```python
from build123d import *

# Parameters (mm, degrees)
BRACKET_BODY_DEPTH      = 56
SLOT_SKETCH_W           = 62
SLOT_SKETCH_H           = 20
SLOT_CUT_DEPTH          = 90.112288715
LUG_A_SKETCH_R          = 32
LUG_A_SKETCH_R_2        = 18
LUG_A_14MM_DEPTH        = 14
SPACER_START            = 2
SPACER_A_SKETCH_R       = 32
SPACER_A_SKETCH_R_2     = 18
SPACER_A_2MM_DEPTH      = 2
HOLE_A_SKETCH_R         = 18
HOLE_A_DEPTH            = 107.244999882
SPACER_B_SKETCH_R       = 32
SPACER_B_SKETCH_R_2     = 18
SPACER_B_2MM_DEPTH      = 2
LUG_B_SKETCH_R          = 32
LUG_B_SKETCH_R_2        = 18
LUG_B_14MM_DEPTH        = 14
PAD_SKETCH_R            = 25
PAD_SKETCH_R_2          = 12.5
PAD_2MM_DEPTH           = 2
HUB_START               = -44
HUB_SKETCH_R            = 25
HUB_SKETCH_R_2          = 12.5
HUB_44MM_DEPTH          = 44
HUB_BORE_SKETCH_R       = 12.5
HUB_BORE_DEPTH          = 44
ARM_35MM_DEPTH          = 35
ARM_SPACER_A_SKETCH_R   = 17.5
ARM_SPACER_A_SKETCH_R_2 = 10
ARM_SPACER_A_2MM_DEPTH  = 2
ARM_START               = -12
ARM_LUG_SKETCH_R        = 17.5
ARM_LUG_SKETCH_R_2      = 10
ARM_LUG_12MM_DEPTH      = 12
ARM_HOLE_SKETCH_R       = 10
ARM_HOLE_DEPTH          = 150.390672563
ARM_SPACER_B_SKETCH_R   = 17.5
ARM_SPACER_B_SKETCH_R_2 = 10
ARM_SPACER_B_2MM_DEPTH  = 2
ARM_START_2             = -14
ARM_EYE_SKETCH_R        = 17.5
ARM_EYE_SKETCH_R_2      = 10
ARM_EYE_14MM_DEPTH      = 14
ARM_SLOT_SKETCH_W       = 12.731987003
ARM_SLOT_SKETCH_H       = 35
ARM_SLOT_10MM_DEPTH     = 10
PIN_START               = -16
PIN_BOSS_SKETCH_R       = 25
PIN_BOSS_16MM_DEPTH     = 16
PIN_BOSS_HOLE_SKETCH_R  = 12.5
PIN_BOSS_HOLE_DEPTH     = 151.168319402


with BuildPart() as part:
    # Bracket Profile Sketch → Bracket Body (new body)
    with BuildSketch(Plane.XY):
        Polygon((0, 0), (17, 0), (17, -48), (31, -48), (31, 12), (9, 12), (9, 62), (-9, 62), (-9, 12), (-31, 12), (-31, -48), (-17, -48), (-17, 0), align=None)
    extrude(amount=-BRACKET_BODY_DEPTH)

    # Slot Sketch → Slot Cut (cut, through all)
    with BuildSketch(Plane.XY):
        with Locations((0, -38)):
            Rectangle(SLOT_SKETCH_W, SLOT_SKETCH_H)
    extrude(amount=-SLOT_CUT_DEPTH, mode=Mode.SUBTRACT)

    # Lug A Sketch → Lug A 14mm (add)
    with BuildSketch(Plane(origin=(31, 0, 0), x_dir=(0, 0, -1), z_dir=(1, 0, 0))):
        with Locations((28, -28)):
            Circle(LUG_A_SKETCH_R)
        with Locations((28, -28)):
            Circle(LUG_A_SKETCH_R_2, mode=Mode.SUBTRACT)
    extrude(amount=-LUG_A_14MM_DEPTH)

    # Spacer A Sketch → Spacer A 2mm (add)
    with BuildSketch(Plane(origin=(31, 0, 0), x_dir=(0, 0, -1), z_dir=(1, 0, 0)).offset(SPACER_START)):
        with Locations(Location((28, -28, 0), (0, 0, 90))):
            Circle(SPACER_A_SKETCH_R)
        with Locations(Location((28, -28, 0), (0, 0, 90))):
            Circle(SPACER_A_SKETCH_R_2, mode=Mode.SUBTRACT)
    extrude(amount=-SPACER_A_2MM_DEPTH)

    # Hole A Sketch → Hole A (cut, through all)
    with BuildSketch(Plane(origin=(31, 0, 0), x_dir=(0, 0, -1), z_dir=(1, 0, 0))):
        with Locations(Location((28, -28, 0), (0, 0, 90))):
            Circle(HOLE_A_SKETCH_R)
    extrude(amount=-HOLE_A_DEPTH, mode=Mode.SUBTRACT)

    # Spacer B Sketch → Spacer B 2mm (add)
    with BuildSketch(Plane.ZY.offset(31)):
        with Locations(Location((-28, -28, 0), (0, 0, 90))):
            Circle(SPACER_B_SKETCH_R)
        with Locations(Location((-28, -28, 0), (0, 0, 90))):
            Circle(SPACER_B_SKETCH_R_2, mode=Mode.SUBTRACT)
    extrude(amount=SPACER_B_2MM_DEPTH)

    # Lug B Sketch → Lug B 14mm (add)
    with BuildSketch(Plane(origin=(-17, 0, 0), x_dir=(0, 0, -1), z_dir=(1, 0, 0))):
        with Locations(Location((28, -28, 0), (0, 0, 90))):
            Circle(LUG_B_SKETCH_R)
        with Locations(Location((28, -28, 0), (0, 0, 90))):
            Circle(LUG_B_SKETCH_R_2, mode=Mode.SUBTRACT)
    extrude(amount=-LUG_B_14MM_DEPTH)

    # Pad Sketch → Pad 2mm (add)
    with BuildSketch(Plane.ZY.offset(9)):
        with Locations(Location((-28, 50, 0), (0, 0, 151.314597986))):
            Circle(PAD_SKETCH_R)
        with Locations(Location((-28, 50, 0), (0, 0, 73.739795292))):
            Circle(PAD_SKETCH_R_2, mode=Mode.SUBTRACT)
    extrude(amount=PAD_2MM_DEPTH)

    # Hub Sketch → Hub 44mm (add)
    with BuildSketch(Plane.ZY.offset(11).offset(HUB_START)):
        with Locations(Location((-28, 50, 0), (0, 0, 270))):
            Circle(HUB_SKETCH_R)
        with Locations(Location((-28, 50, 0), (0, 0, 270))):
            Circle(HUB_SKETCH_R_2, mode=Mode.SUBTRACT)
    extrude(amount=HUB_44MM_DEPTH)

    # Hub Bore Sketch → Hub Bore (cut)
    with BuildSketch(Plane.ZY.offset(9).offset(HUB_START)):
        with Locations(Location((-28, 50, 0), (0, 0, 270))):
            Circle(HUB_BORE_SKETCH_R)
    extrude(amount=HUB_BORE_DEPTH, mode=Mode.SUBTRACT)

    # Arm Profile Sketch → Arm 35mm (add)
    with BuildSketch(Plane(origin=(0, 62, 0), x_dir=(1, 0, 0), z_dir=(0, 1, 0))):
        Polygon((3.731987003, 49.931712199), (3.731987003, 79.931712199), (-8.268012997, 79.931712199), (-8.268012997, 104.931712199), (3.731987003, 104.931712199), (3.731987003, 92.431712199), (18.731987003, 92.431712199), (18.731987003, 104.931712199), (30.731987003, 104.931712199), (30.731987003, 79.931712199), (18.731987003, 79.931712199), (18.731987003, 49.931712199), align=None)
    extrude(amount=-ARM_35MM_DEPTH)

    # Arm Spacer A Sketch → Arm Spacer A 2mm (add)
    with BuildSketch(Plane.ZY.offset(8.268012997)):
        with Locations(Location((-104.931712199, 44.5, 0), (0, 0, 270))):
            Circle(ARM_SPACER_A_SKETCH_R)
        with Locations(Location((-104.931712199, 44.5, 0), (0, 0, 90))):
            Circle(ARM_SPACER_A_SKETCH_R_2, mode=Mode.SUBTRACT)
    extrude(amount=ARM_SPACER_A_2MM_DEPTH)

    # Arm Lug Sketch → Arm Lug 12mm (add)
    with BuildSketch(Plane.ZY.offset(8.268012997).offset(ARM_START)):
        with Locations(Location((-104.931712199, 44.5, 0), (0, 0, 90))):
            Circle(ARM_LUG_SKETCH_R)
        with Locations(Location((-104.931712199, 44.5, 0), (0, 0, 90))):
            Circle(ARM_LUG_SKETCH_R_2, mode=Mode.SUBTRACT)
    extrude(amount=ARM_LUG_12MM_DEPTH)

    # Arm Hole Sketch → Arm Hole (cut, through all)
    with BuildSketch(Plane.ZY.offset(8.268012997)):
        with Locations((-104.931712199, 44.5)):
            Circle(ARM_HOLE_SKETCH_R)
    extrude(amount=-ARM_HOLE_DEPTH, mode=Mode.SUBTRACT)

    # Arm Spacer B Sketch → Arm Spacer B 2mm (add)
    with BuildSketch(Plane(origin=(30.731987003, 0, 0), x_dir=(0, 0, -1), z_dir=(1, 0, 0))):
        with Locations(Location((104.931712199, 44.5, 0), (0, 0, 90))):
            Circle(ARM_SPACER_B_SKETCH_R)
        with Locations(Location((104.931712199, 44.5, 0), (0, 0, 180))):
            Circle(ARM_SPACER_B_SKETCH_R_2, mode=Mode.SUBTRACT)
    extrude(amount=ARM_SPACER_B_2MM_DEPTH)

    # Arm Eye Sketch → Arm Eye 14mm (add)
    with BuildSketch(Plane(origin=(32.731987003, 0, 0), x_dir=(0, 0, -1), z_dir=(1, 0, 0)).offset(ARM_START_2)):
        with Locations(Location((104.931712199, 44.5, 0), (0, 0, 90))):
            Circle(ARM_EYE_SKETCH_R)
        with Locations(Location((104.931712199, 44.5, 0), (0, 0, 180))):
            Circle(ARM_EYE_SKETCH_R_2, mode=Mode.SUBTRACT)
    extrude(amount=ARM_EYE_14MM_DEPTH)

    # Arm Slot Sketch → Arm Slot 10mm (cut)
    with BuildSketch(Plane(origin=(0, 0, -56), x_dir=(-1, 0, 0), z_dir=(0, 0, -1))):
        with Locations((2.634006498, 44.5)):
            Rectangle(ARM_SLOT_SKETCH_W, ARM_SLOT_SKETCH_H)
    extrude(amount=-ARM_SLOT_10MM_DEPTH, mode=Mode.SUBTRACT)

    # Pin Boss Sketch → Pin Boss 16mm (add)
    with BuildSketch(Plane.ZY.offset(11).offset(PIN_START)):
        with Locations(Location((-28, 50, 0), (0, 0, 270))):
            Circle(PIN_BOSS_SKETCH_R)
    extrude(amount=PIN_BOSS_16MM_DEPTH)

    # Pin Boss Hole Sketch → Pin Boss Hole (cut, through all)
    with BuildSketch(Plane.ZY.offset(11)):
        with Locations(Location((-28, 50, 0), (0, 0, 270))):
            Circle(PIN_BOSS_HOLE_SKETCH_R)
    extrude(amount=-PIN_BOSS_HOLE_DEPTH, mode=Mode.SUBTRACT)


solid = part.part
```
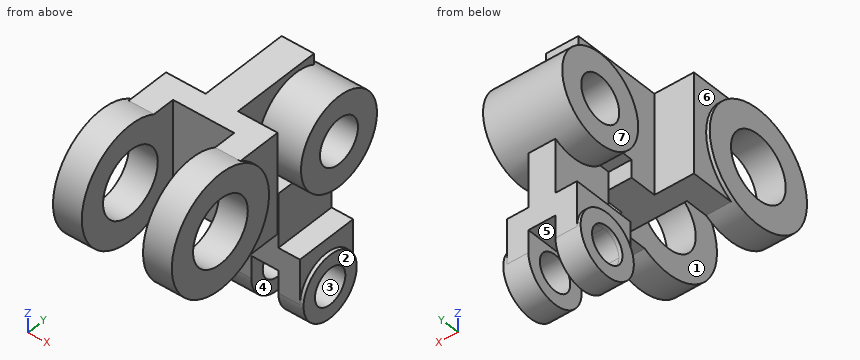
Design review of the part built by this model. Coordinates are the model's own, in mm. Face numbers are marked on the shaded views. A direction names the side the tool comes from. Give positions to 0.01 mm unless a question says otherwise; leave off trailing zeros. Loops run counter-clockwise (first coordinate to the right, second up) from the corner with the lowest first, then second, coordinate; pieces in that order, holes last. Notation, with made-up numbers: M 49,50.5 L 82,50.5 A21 ccw 82,86.5 Z; hole C 77.5,12 d7. An arc over 180 degrees is marked long. Return JSON: item names as keys, results as strings. Group by question number.
Item 1: We need section C-C (x = -20). Give the boundary of the cut face in (y, z), and give its area (3 significant figures).
Item 2: We need section A-A (y = -28). Give the boundary of the cut face in (x, z), and give its area (3 significant figures).
Item 3: We need section D-D (z = -63). Give the boundary of the cut face in (x, y).
Item 4: We need section B-B (z = -102.5). Give the boundary of the cut face in (x, y), and give its area (3 significant figures).
Item 5: Insertion check: pin 1 Ø20 at (y, z) = (48.5, -92.5) entering from +X; pin 2 Ø11.5 at (x, z) = (9.5, -89.5) entering from -Y; pin 3 Ø5 at (x, z) = (-5, -53) entering from +Y; pin 4 Ø16 at (y, z) = (44.5, -104.93) entering from -X. Each pin has a flat end and moves straight along its axis. Give the tip position at first contact, or say it passes through.
Item 6: Mouldability with a two-part tool opening along X and no side actions: class the marked faces 1, 2, 3 and 4 as released by +X, released by -X, zero draft, split by the parting line, or undercut.
Item 7: Tool access review of the marked faces 5, 6 and 7: name each direction out of +Z, -Z, +X, -X, +Y, -Y from which nothing blocks a thin tool from reaching the whole face with its end or side.
Item 8: For probe 1 along Y at (x, z) = (-27.25, -28); probe 2 along X at (y, z) = (29.5, -94); probe 3 along Z at (x, y) = (-25, -28), list the stretches that pass through material, from the lowest coordinate up.
Output:
{
 "1": {"outline": "M -12.51,-56 L 12,-56 L 12,0 L -12.51,0 A32 ccw long Z; hole C -28,-28 d36", "area": "2,910 mm^2"},
 "2": {"outline": "M -33,-60 L -17,-60 L -17,-46 L -33,-46 Z; M -33,-10 L -17,-10 L -17,4 L -33,4 Z; M 17,-60 L 33,-60 L 33,-46 L 17,-46 Z; M 17,-10 L 33,-10 L 33,4 L 17,4 Z", "area": "896 mm^2"},
 "3": {"outline": "M 3.73,27 L 18.73,27 L 18.73,62 L 3.73,62 Z"},
 "4": {"outline": "M -10.27,27.17 L -8.27,27.17 L -8.27,27 L 3.73,27 L 3.73,34.8 L -10.27,34.8 Z; M -10.27,54.2 L 3.73,54.2 L 3.73,62 L -8.27,62 L -8.27,61.83 L -10.27,61.83 Z; M 18.73,27 L 30.73,27 L 30.73,27.17 L 32.73,27.17 L 32.73,34.8 L 18.73,34.8 Z; M 18.73,54.2 L 32.73,54.2 L 32.73,61.83 L 30.73,61.83 L 30.73,62 L 18.73,62 Z", "area": "435 mm^2"},
 "5": {"pin 1": "stops at x = 32.73", "pin 2": "stops at y = 27", "pin 3": "stops at y = 60.9", "pin 4": "passes through"},
 "6": {"face 1": "undercut", "face 2": "released by +X", "face 3": "zero draft", "face 4": "undercut"},
 "7": {"face 5": "-Z, +Y, -Y", "face 6": "-X, +Y", "face 7": "+Z, -Z, -X, +Y"},
 "8": {"probe 1": "y = -60 to -46, -10 to 12", "probe 2": "x = -8.27 to 3.73, 18.73 to 30.73", "probe 3": "z = -60 to -46, -10 to 4"}
}
